from build123d import *

# Parameters (mm, degrees)
SKETCH1_R           = 3
BOSS_EXTRUDE1_DEPTH = 10
BOSS_EXTRUDE2_DEPTH = 6


with BuildPart() as part:
    # Sketch1 → Boss-Extrude1 (new body)
    with BuildSketch(Plane.XY):
        Circle(SKETCH1_R)
    extrude(amount=BOSS_EXTRUDE1_DEPTH)

    # Sketch2 → Boss-Extrude2 (add)
    with BuildSketch(Plane.XY.offset(10)):
        Polygon((-5.196152423, -3), (0, -6), (5.196152423, -3), (5.196152423, 3), (0, 6), (-5.196152423, 3), align=None)
    extrude(amount=BOSS_EXTRUDE2_DEPTH)


solid = part.part
Geometry check sheet. Reference: the model listing, model coordinates, mm. A direction names the side the tool comes from. Give positions to 0.01 mm unless a question says otherwise; leave off trailing zeros. Write each loop counter-clockwise with the first axis right and the second up, starting at its lowest first coordinate (ties: lowest second). Pieces come first, ordered by that corner, then holes. Notation, with made-up numbers: (58, 78) - (100, 78) arc R26 cw to (100, 108) - close; hole circle Ø9 at (51.25, 11). An arc over 180 degrees is marked (long way). Put each result on its own line as item: value.
1. Sectioned sample at A-A, the plane y = 0. Enter the section's corners in (x, z).
Ans:
outline: (-5.2, 10) - (-3, 10) - (-3, 0) - (3, 0) - (3, 10) - (5.2, 10) - (5.2, 16) - (-5.2, 16) - close
2. Sectioned sample at D-D, the plane z = 3. Enter the section's corners in (x, y).
Ans:
outline: circle Ø6 at (0, 0)
3. Go/stop test with flat-tipped pins: pin 1 (1.5 mm diameter, centred on y = 3, z = 7, fed in from -X); pin 2 (4 mm diameter, centred on x = 1.5, z = 9, fed in from +Y); pin 3 (1 mm diameter, centred on x = -4, z = 10.5, fed in from -Y). Record where each tip stops, or that it passes through.
Ans:
pin 1: stops at x = -1.98
pin 2: stops at y = 6
pin 3: stops at y = -3.98
4. Sectioned sample at B-B, the plane z = 13. Enter the section's corners in (x, y).
Ans:
outline: (-5.2, -3) - (0, -6) - (5.2, -3) - (5.2, 3) - (0, 6) - (-5.2, 3) - close
5. Set-up check for faces 1 (the flat face through (2.6, 4.5, 13)), 2 (the cylindrical face through (-3, 0, 5)): record each of +Z, -Z, +X, -X, +Y, -Y from which the full face is reachable in a straight line by a thin tool's end or side.
Ans:
face 1: +Z, -Z, +X, +Y
face 2: -Z
6. Sectioned sample at C-C, the plane x = -2.75. Enter the section's corners in (y, z), plus the area to 3 significant figures.
Ans:
outline: (-4.41, 10) - (-1.2, 10) - (-1.2, 0) - (1.2, 0) - (1.2, 10) - (4.41, 10) - (4.41, 16) - (-4.41, 16) - close
area: 76.9 mm²
7. Thickness scan on line 1 (Z direction, x = 4.75, y = -0.5); line 2 (Y direction, x = -4.5, z = 12.5); line 3 (X direction, y = -4.5, z = 15.25). Record the ranges inside material, lowest first.
Ans:
line 1: z = 10 to 16
line 2: y = -3.4 to 3.4
line 3: x = -2.6 to 2.6
